Geometry check sheet. Reference: the model listing, model coordinates, mm. A direction names the side the tool comes from. Give positions to 0.01 mm unless a question says otherwise; leave off trailing zeros. Order: outer loops, then holes, each group sorted by start corner. A loop starts at its lowest first (then second) coordinate and runs counter-clockwise, first axis right, second up.
from build123d import *

# Parameters (mm, degrees)
BASE_BLOCK_DEPTH            = 55
HOLES_SKETCH_R              = 7
HOLES_2X_14_DEPTH           = 22
ARM_RISER_SKETCH_W          = 15
ARM_RISER_SKETCH_H          = 12
ARM_RISER_DEPTH             = 40
OFFSET_ARM_DEPTH            = 15
SLOTTED_CLAMP_BLOCK_DEPTH   = 35
CLAMP_BLOCK_EXTENSION_DEPTH = 15


with BuildPart() as part:
    # Base Block Profile → Base Block (new body)
    with BuildSketch(Plane.XY):
        with BuildLine():
            Line((50, -10), (50, -35))
            Line((50, -35), (32, -35))
            Line((32, -35), (32, -20))
            Line((32, -20), (0, -20))
            Line((0, -20), (0, 0))
            Line((0, 0), (40, 0))
            ThreePointArc((40, 0), (47.071067812, -2.928932188), (50, -10))
        make_face()
    extrude(amount=BASE_BLOCK_DEPTH)

    # Holes Sketch → Holes 2x_14 (cut)
    with BuildSketch(Plane(origin=(0, 0, 0), x_dir=(1, 0, 0), z_dir=(0, 1, 0))):
        with Locations(Location((20, -15, 0), (0, 0, 270))):
            Circle(HOLES_SKETCH_R)
        with Locations(Location((20, -40, 0), (0, 0, 270))):
            Circle(HOLES_SKETCH_R)
    extrude(amount=-HOLES_2X_14_DEPTH, mode=Mode.SUBTRACT)

    # Arm Riser Sketch → Arm Riser (add)
    with BuildSketch(Plane.ZY):
        with Locations((32.5, -6)):
            Rectangle(ARM_RISER_SKETCH_W, ARM_RISER_SKETCH_H)
    extrude(amount=ARM_RISER_DEPTH)

    # Offset Arm Profile → Offset Arm (add)
    with BuildSketch(Plane.XY.offset(40)):
        with BuildLine():
            Line((-40, -12), (-52, -12))
            ThreePointArc((-52, -12), (-56.242640687, -10.242640687), (-58, -6))
            Line((-58, -6), (-58, 40))
            Line((-58, 40), (-121, 40))
            Line((-121, 40), (-121, 50))
            Line((-121, 50), (-71, 50))
            Line((-71, 50), (-71, 55))
            Line((-71, 55), (-40, 55))
            Line((-40, 55), (-40, 0))
            Line((-40, 0), (0, 0))
            Line((0, 0), (0, -12))
            Line((0, -12), (-40, -12))
        make_face()
    extrude(amount=-OFFSET_ARM_DEPTH)

    # Slotted Clamp Block Profile → Slotted Clamp Block (add)
    with BuildSketch(Plane.XY.offset(40)):
        Polygon((-121, 50), (-71, 50), (-71, 75), (-86, 75), (-86, 60), (-106, 60), (-106, 75), (-121, 75), align=None)
    extrude(amount=-SLOTTED_CLAMP_BLOCK_DEPTH)

    # Clamp Block Extension Profile → Clamp Block Extension (add)
    with BuildSketch(Plane.XY.offset(40)):
        Polygon((-121, 75), (-121, 50), (-71, 50), (-71, 75), (-86, 75), (-86, 60), (-106, 60), (-106, 75), align=None)
    extrude(amount=CLAMP_BLOCK_EXTENSION_DEPTH)


solid = part.part
Item 1: Sectioned sample at A-A (z = 15). Enter the section's corners in (x, y).
Reported:
outline: (-121, 50) - (-71, 50) - (-71, 75) - (-86, 75) - (-86, 60) - (-106, 60) - (-106, 75) - (-121, 75) - close; (0, -20) - (13, -20) - (13, 0) - (0, 0) - close; (27, -20) - (32, -20) - (32, -35) - (50, -35) - (50, -10) arc R10 ccw to (40, 0) - (27, 0) - close
Item 2: Set-up check for faces 1 (the flat face through (-86, 68, 30)), 2 (the flat face through (-26, -12, 33)), 3 (the flat face through (-96, 50, 47)): record each of +Z, -Z, +X, -X, +Y, -Y from which the full face is reachable in a straight line by a thin tool's end or side.
Reported:
face 1: +Z, -Z, +Y
face 2: +Z, -Z, -X, -Y
face 3: +Z, +X, -X, -Y
Item 3: Scan lines: L1, parallel to X at y = -15, z = 40; L2, parallel to X at y = 67.5, z = 39.5; L3, parallel to Y at x = 38.5, z = 16. Record each from-to range of solid material in increasing order.
Reported:
L1: x = 0 to 13, 27 to 50
L2: x = -121 to -106, -86 to -71
L3: y = -35 to 0
Item 4: Sectioned sample at D-D (x = -21). Enter the section's corners in (y, z), and give its area (3 significant figures).
Reported:
outline: (-12, 25) - (0, 25) - (0, 40) - (-12, 40) - close
area: 180 mm2
Item 5: Draft check along X on faces 4 (the flat face through (-106, 67, 30)), 5 (the flat face through (32, -28, 27)), 6 (the flat face through (41, -35, 27)), 7 (the cylindrical face through (13.79, -9.86, 43.23)). Enter one of: released by +X, released by -X, zero draft, split by the parting line, or undercut.
Reported:
face 4: undercut
face 5: released by -X
face 6: zero draft
face 7: undercut
Item 6: Sectioned sample at C-C (x = -101.5). Enter the section's corners in (y, z).
Reported:
outline: (40, 25) - (50, 25) - (50, 5) - (60, 5) - (60, 55) - (50, 55) - (50, 40) - (40, 40) - close
Item 7: Gauge pin test, flat ends, axial feed: pin 1 (4.5 mm diameter, centred on y = -24, z = 40, fed in from -X); pin 2 (16.5 mm diameter, centred on y = 28.5, z = 32, fed in from +X); pin 3 (7.5 mm diameter, centred on x = -83.5, z = 46, fed in from -Y); pin 4 (11 mm diameter, centred on x = 20, z = 40, fed in from -Y). Record the tip position at first contact, or that the pin passes through.
Reported:
pin 1: stops at x = 32
pin 2: stops at x = -40
pin 3: stops at y = 50
pin 4: passes through
Item 8: Sectioned sample at B-B (x = 20). Enter the section's corners in (y, z).
Reported:
outline: (-20, 0) - (0, 0) - (0, 8) - (-20, 8) - close; (-20, 22) - (0, 22) - (0, 33) - (-20, 33) - close; (-20, 47) - (0, 47) - (0, 55) - (-20, 55) - close
